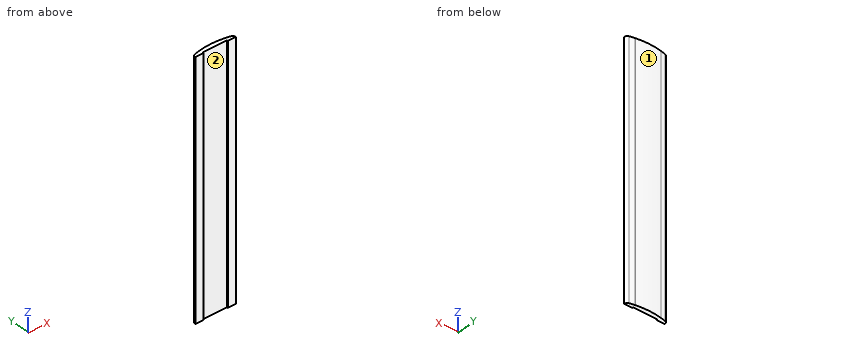
```python
from build123d import *

# Parameters (mm, degrees)
EXTRUDE_1_DEPTH = 575
FILLET_1_R      = 0.3


with BuildPart() as part:
    # 草图1 → 凸台-拉伸1 (new, symmetric)
    with BuildSketch(Plane.XY):
        with BuildLine():
            Line((94, 0), (56.7, 0))
            ThreePointArc((56.7, 0), (56.558578644, 0.058578644), (56.5, 0.2))
            Line((56.5, 0.2), (56.5, 4.5))
            Line((56.5, 4.5), (-56.5, 4.5))
            Line((-56.5, 4.5), (-56.5, 0.2))
            ThreePointArc((-56.5, 0.2), (-56.558578644, 0.058578644), (-56.7, 0))
            Line((-56.7, 0), (-94, 0))
            ThreePointArc((-94, 0), (-91.314648859, 8.987866196), (-83.557929261, 14.262916014))
            ThreePointArc((-83.557929261, 14.262916014), (-72.015896085, 17.05846092), (-60.38087895, 19.437531623))
            ThreePointArc((-60.38087895, 19.437531623), (-60.316820101, 19.428115404), (-60.271957046, 19.381430208))
            ThreePointArc((-60.271957046, 19.381430208), (-59.945537065, 19.213061927), (-59.70074969, 19.486881253))
            ThreePointArc((-59.70074969, 19.486881253), (-59.675512901, 19.546507637), (-59.619038631, 19.578175571))
            ThreePointArc((-59.619038631, 19.578175571), (-59.500070371, 19.599971741), (-59.381094143, 19.621724372))
            ThreePointArc((-59.381094143, 19.621724372), (-59.317064562, 19.612111154), (-59.272345321, 19.565288181))
            ThreePointArc((-59.272345321, 19.565288181), (-58.946444781, 19.395916638), (-58.700816303, 19.668981709))
            ThreePointArc((-58.700816303, 19.668981709), (-58.675396224, 19.728530183), (-58.618824811, 19.760024254))
            ThreePointArc((-58.618824811, 19.760024254), (0, 25), (58.618824811, 19.760024254))
            ThreePointArc((58.618824811, 19.760024254), (58.675396224, 19.728530183), (58.700816303, 19.668981709))
            ThreePointArc((58.700816303, 19.668981709), (58.946444781, 19.395916638), (59.272345321, 19.565288181))
            ThreePointArc((59.272345321, 19.565288181), (59.317064562, 19.612111154), (59.381094143, 19.621724372))
            ThreePointArc((59.381094143, 19.621724372), (59.500070371, 19.599971741), (59.619038631, 19.578175571))
            ThreePointArc((59.619038631, 19.578175571), (59.675512901, 19.546507637), (59.70074969, 19.486881253))
            ThreePointArc((59.70074969, 19.486881253), (59.945537065, 19.213061927), (60.271957046, 19.381430208))
            ThreePointArc((60.271957046, 19.381430208), (60.316820101, 19.428115404), (60.38087895, 19.437531623))
            ThreePointArc((60.38087895, 19.437531623), (72.015896085, 17.05846092), (83.557929261, 14.262916014))
            ThreePointArc((83.557929261, 14.262916014), (91.314648859, 8.987866196), (94, 0))
        make_face()
    extrude(amount=EXTRUDE_1_DEPTH, both=True)

    # 圆角1
    fillet_1_edges = [part.edges().sort_by_distance(p)[0] for p in [
        (94, 0, 0),
        (-94, 0, 0),
    ]]
    fillet(fillet_1_edges, radius=FILLET_1_R)


solid = part.part
```
Geometry check sheet. Reference: the model listing, model coordinates, mm. Face numbers are marked on the shaded views. Round coordinates to 2 decimals unless told otherwise and drop trailing zeros. Order: outer loops, then holes, each group sorted by start corner. A loop starts at its lowest first (then second) coordinate and runs counter-clockwise, first axis right, second up. Notation, with made-up numbers: (57, -33.5) - (87, -33.5) arc R15 ccw to (87, -6.5) - close; hole circle Ø9 at (53.25, -0.5). An arc over 180 degrees is marked (long way). Use a Markdown table: item, result. Add a question column.
1) Thickness scan on line 1 along X through (y, z) = (19.5, -275.5); line 2 along X through (y, z) = (3.75, 76.5); line 3 along X through (y, z) = (1.5, -347). Record the ranges inside material, lowest first.
2) Section check A-A (z = -412). Record the cut outline in (x, y).
3) Mould release check, pull along X, two halves, no side actions. Record for the marked faces 1 and 2: released by +X, released by -X, zero draft, split by the parting line, or undercut.
4) Gauge pin test, flat ends, axial feed: P1, Ø4, axis at x = -13, z = -226.5, coming from the +Y side; P2, Ø2, axis at y = 2.5, z = -36, coming from the +X side. Record the tip position at first contact, or that the pin passes through.
5) Section check C-C (y = 10.5). Record the cut outline in (x, z), then the cut area to 3 significant figures.
6) Section check B-B (x = 0). Record the cut outline in (y, z), then the cut area to 3 significant figures.
Established:
| question | item | result |
|---|---|---|
| 1 | line 1 | -59.7 to -59.23, -58.77 to 58.77, 59.23 to 59.7 |
| 1 | line 2 | -93.69 to -56.5, 56.5 to 93.69 |
| 1 | line 3 | -94 to -56.5, 56.5 to 94 |
| 2 | outline | (-94.01, 0.29) arc R0.3 ccw to (-93.71, 0) - (-56.7, 0) arc R0.2 ccw to (-56.5, 0.2) - (-56.5, 4.5) - (56.5, 4.5) - (56.5, 0.2) arc R0.2 ccw to (56.7, 0) - (93.71, 0) arc R0.3 ccw to (94.01, 0.29) arc R14 ccw to (83.56, 14.26) arc R330.5 ccw to (60.38, 19.44) arc R0.1 ccw to (60.27, 19.38) arc R0.3 cw to (59.7, 19.49) arc R0.1 ccw to (59.62, 19.58) arc R330.5 ccw to (59.38, 19.62) arc R0.1 ccw to (59.27, 19.57) arc R0.3 cw to (58.7, 19.67) arc R0.1 ccw to (58.62, 19.76) arc R330.5 ccw to (-58.62, 19.76) arc R0.1 ccw to (-58.7, 19.67) arc R0.3 cw to (-59.27, 19.57) arc R0.1 ccw to (-59.38, 19.62) arc R330.5 ccw to (-59.62, 19.58) arc R0.1 ccw to (-59.7, 19.49) arc R0.3 cw to (-60.27, 19.38) arc R0.1 ccw to (-60.38, 19.44) arc R330.5 ccw to (-83.56, 14.26) arc R14 ccw to start |
| 3 | face 1 | split by the parting line |
| 3 | face 2 | undercut |
| 4 | P1 | y = 24.82 |
| 4 | P2 | x = 94 |
| 5 | outline | (-90.03, -575) - (90.03, -575) - (90.03, 575) - (-90.03, 575) - close |
| 5 | area | 207,000 mm2 |
| 6 | outline | (4.5, -575) - (25, -575) - (25, 575) - (4.5, 575) - close |
| 6 | area | 23,600 mm2 |
